```python
from build123d import *

# Parameters (mm, degrees)
BASEKEY_DEPTH = 6
CHAMFER1_SIZE = 0.8


with BuildPart() as part:
    # Sketch1 → BaseKey (new, symmetric)
    with BuildSketch(Plane.XY):
        with BuildLine():
            Line((-36, 10), (0, 10))
            ThreePointArc((0, 10), (10, 0), (0, -10))
            Line((0, -10), (-36, -10))
            ThreePointArc((-36, -10), (-46, 0), (-36, 10))
        make_face()
    extrude(amount=BASEKEY_DEPTH, both=True)

    # Chamfer1
    chamfer1_edges = [part.edges().sort_by_distance(p)[0] for p in [
        (10, 0, 6),
        (-18, 10, 6),
        (-46, 0, 6),
        (-18, 10, -6),
        (10, 0, -6),
        (-18, -10, -6),
        (-46, 0, -6),
        (-18, -10, 6),
    ]]
    chamfer(chamfer1_edges, length=CHAMFER1_SIZE)


solid = part.part
```
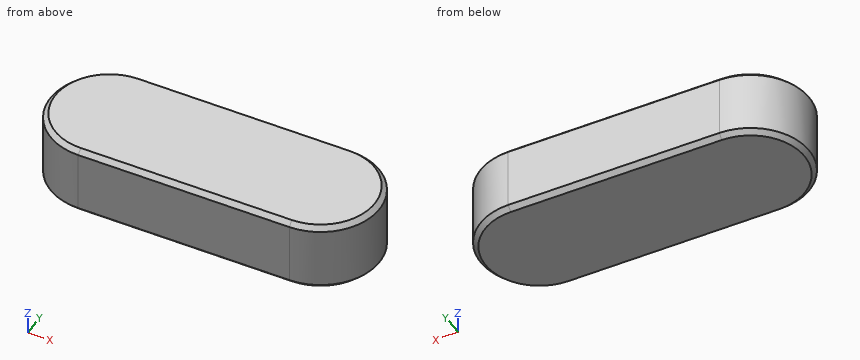
Model file for the job. Use its own axes, mm. Round coordinates to 2 decimals unless told otherwise and drop trailing zeros. Write each loop counter-clockwise with the first axis right and the second up, starting at its lowest first coordinate (ties: lowest second). Pieces come first, ordered by that corner, then holes. Notation, with made-up numbers: (81, 78.5) - (129, 78.5) arc R16 ccw to (129, 101.5) - close; hole circle Ø10 at (39.5, -9). An arc over 180 degrees is marked (long way). Use CSV: the item, a comma, the result in double quotes. Start each with the question number.
Item 1: Drill centre lines: L1, parallel to X at y = 0, z = 2.25; L2, parallel to X at y = 2.75, z = 3.5; L3, parallel to Y at x = -40.5, z = -3.25. Where is each one in solid material? Low to high. Write a range as [from, to].
Item 2: Pin check, flat tips, straight feed: P1, Ø5, axis at y = 5, z = -3.5, coming from the -X side; P2, Ø1.5, axis at x = 2, z = 4, coming from the -Y side; P3, Ø6, axis at y = -8, z = 0, coming from the -X side. Stop position of each tip, or through.
Item 3: Band-saw the part on A-A (z = -2). Write the cut outline in (x, y), and give its area (3 significant figures).
Checked values:
1,L1,"x = [-46, 10]"
1,L2,"x = [-45.61, 9.61]"
1,L3,"y = [-8.93, 8.93]"
2,P1,"stops at x = -45.68"
2,P2,"stops at y = -9.92"
2,P3,"stops at x = -44.66"
3,outline,"(-36, -10) - (0, -10) arc R10 ccw to (0, 10) - (-36, 10) arc R10 ccw to start"
3,area,"1,030 mm²"
